from build123d import *

# Parameters (mm, degrees)
BASE_PLATE_DEPTH     = 5
PIN_CIRCLES_SKETCH_R = 5
PINS_2X_10_DEPTH     = 15


with BuildPart() as part:
    # Plate Outline Sketch → Base Plate (new body)
    with BuildSketch(Plane.XY):
        with BuildLine():
            Line((-27.5, 15), (27.5, 15))
            ThreePointArc((27.5, 15), (42.5, 0), (27.5, -15))
            Line((27.5, -15), (-27.5, -15))
            ThreePointArc((-27.5, -15), (-42.5, 0), (-27.5, 15))
        make_face()
    extrude(amount=BASE_PLATE_DEPTH)

    # Pin Circles Sketch → Pins 2xØ10 (add)
    with BuildSketch(Plane.XY.offset(5)):
        with Locations((-27.5, 0)):
            Circle(PIN_CIRCLES_SKETCH_R)
        with Locations((27.5, 0)):
            Circle(PIN_CIRCLES_SKETCH_R)
    extrude(amount=PINS_2X_10_DEPTH)


solid = part.part
Read the model definition and answer for the solid it produces. Units are mm, in the model's axes. A direction names the side the tool comes from. Coordinates: 2 decimals unless noted, no trailing zeros. Write each loop counter-clockwise with the first axis right and the second up, starting at its lowest first coordinate (ties: lowest second). Pieces come first, ordered by that corner, then holes. Notation, with made-up numbers: (69.5, 46) - (77.5, 46) arc R20 cw to (77.5, 65) - close; hole circle Ø8 at (52.25, 29.25). An arc over 180 degrees is marked (long way). One line per question, with ' | ' between items.
Q1. Find section A-A, the plane z = 17.5. Write down the section's boundary in (x, y).
Result set:
outline: circle Ø10 at (-27.5, 0); circle Ø10 at (27.5, 0)
Q2. Find section C-C, the plane x = -29.5. Write down the section's boundary in (y, z), plus the area to 3 significant figures.
Result set:
outline: (-14.87, 0) - (14.87, 0) - (14.87, 5) - (4.58, 5) - (4.58, 20) - (-4.58, 20) - (-4.58, 5) - (-14.87, 5) - close | area: 286 mm^2
Q3. Consider L1, parallel to X at y = 1, z = 18.5; L2, parallel to X at y = -3, z = 7.75; L3, parallel to Z at x = 5, y = 3.5. Determine where each line is inside the solid, lowest interval first. Write a range as [from, to].
Result set:
L1: [-32.4, -22.6], [22.6, 32.4] | L2: [-31.5, -23.5], [23.5, 31.5] | L3: [0, 5]
Q4. Each of these flat-tipped pins is pushed along its axis until it touches: P1, Ø5, axis at y = -2, z = 14.5, coming from the -X side; P2, Ø5, axis at x = 20.5, y = -6.5, coming from the +Z side; P3, Ø1.5, axis at x = -13.5, y = 1.5, coming from the -Z side; P4, Ø1, axis at x = -32, z = 7, coming from the +Y side. Where does it stop, or does it pass through?
Result set:
P1: x = -32.5 | P2: z = 5 | P3: z = 0 | P4: y = 3
Q5. Find section B-B, the plane y = 0. Write down the section's boundary in (x, z), plus the area to 3 significant figures.
Result set:
outline: (-42.5, 0) - (42.5, 0) - (42.5, 5) - (32.5, 5) - (32.5, 20) - (22.5, 20) - (22.5, 5) - (-22.5, 5) - (-22.5, 20) - (-32.5, 20) - (-32.5, 5) - (-42.5, 5) - close | area: 725 mm^2
Q6. For faces 1 (the cylindrical face through (-42.496, -0.33, 2.465)), 2 (the cylindrical face through (22.505, 0.22, 12.395)), determine the directions among +Z, -Z, +X, -X, +Y, -Y from which every point of the face is accessible in a straight line to the end or side of a thin tool.
Result set:
face 1: +Z, -Z, -X | face 2: +Z
Q7. Find section D-D, the plane y = 9. Write down the section's boundary in (x, z), plus the area to 3 significant figures.
Result set:
outline: (-39.5, 0) - (39.5, 0) - (39.5, 5) - (-39.5, 5) - close | area: 395 mm^2
